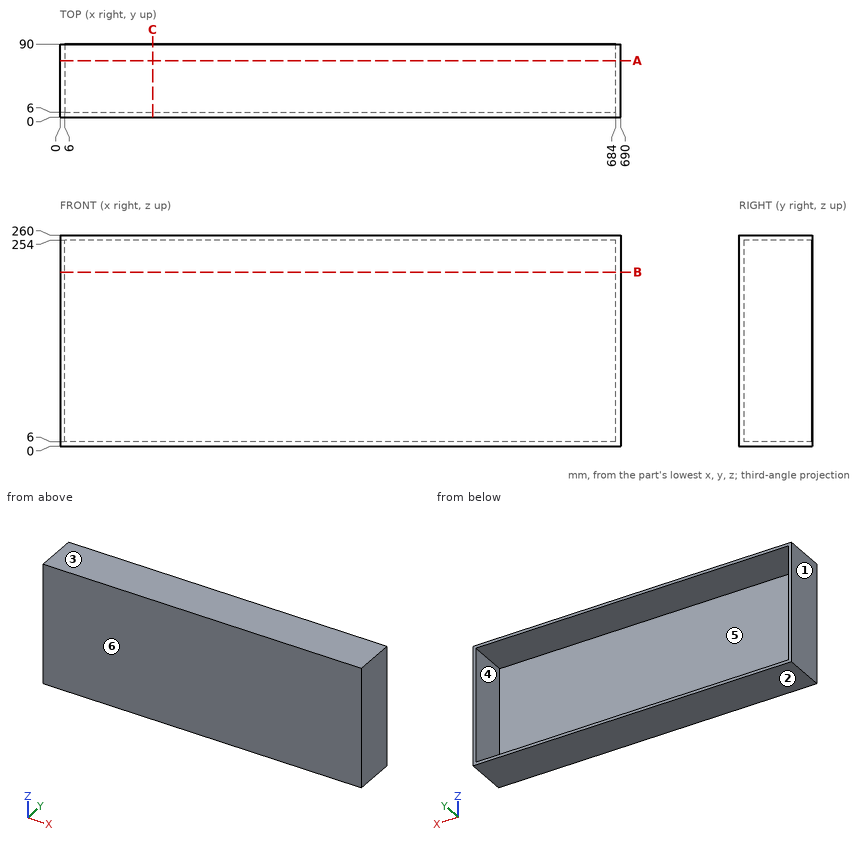
Here's the drawing with two shaded views (mm, measured from the low corner). I have some questions. A direction names the side the tool comes from. Round coordinates to 2 decimals unless told otherwise and drop trailing zeros. Loops run counter-clockwise (first coordinate to the right, second up) from the corner with the lowest first, then second, coordinate; pieces in that order, holes last. Notation, with made-up numbers: M -27,35.25 L 3,35.25 A26 cw 3,53.25 Z; hole C -29.5,48 d10. An arc over 180 degrees is marked long. Answer as a JSON object with one key per item and string values. Group by question number.
Q1. Please list where these lines run through material, in increasing order: L1, parallel to X at y = 14.5, z = 233; L2, parallel to Z at x = 400.5, y = 75; L3, parallel to Y at x = 208.5, z = 248.
Q2. Imagine slicing it at C-C, the plane x = 114. Please give me the cut outline in (y, z).
Q3. Imagine slicing it at A-A, the plane y = 69.5. Please give me the cut outline in (x, z).
Q4. We'd pull the mould along Z, two halves only. Please class the marked faces 1, 2, 3 and 4: +Z half, -Z half, draft (parallel to the pull), parting line (faces both ways), or undercut.
Q5. Imagine slicing it at B-B, the plane z = 214.5. Please give me the cut outline in (x, y), then the cut area to 3 significant figures.
Q6. On a 3-axis mill with a long thin cutter (end or side, diameter ignored), from which of +Z, -Z, +X, -X, +Y, -Y can I reach the whole of each face in a straight line? I mean the marked faces 5 and 6. Say none if no direction works.
Q7. Will this pin go through, and if not, where does the flat tip stop? pin 1 (12 mm diameter, centred on x = 245.5, z = 76, fed in from +Y).
Findings:
{
 "1": {"L1": "x = 0 to 6, 684 to 690", "L2": "z = 0 to 6, 254 to 260", "L3": "y = 0 to 6"},
 "2": {"outline": "M 0,0 L 90,0 L 90,6 L 6,6 L 6,254 L 90,254 L 90,260 L 0,260 Z"},
 "3": {"outline": "M 0,0 L 690,0 L 690,260 L 0,260 Z; hole M 6,6 L 684,6 L 684,254 L 6,254 Z"},
 "4": {"face 1": "draft", "face 2": "-Z half", "face 3": "+Z half", "face 4": "undercut"},
 "5": {"outline": "M 0,0 L 690,0 L 690,90 L 684,90 L 684,6 L 6,6 L 6,90 L 0,90 Z", "area": "5,150 mm2"},
 "6": {"face 5": "+Y", "face 6": "+Z, -Z, +X, -X, -Y"},
 "7": {"pin 1": "stops at y = 6"}
}
